Input: dimensioned drawing with shaded views. Units: mm. Origin: part minimum x, y, z. A direction names the side the tool comes from. Coordinates: 2 decimals unless noted, no trailing zeros. Order: outer loops, then holes, each group sorted by start corner. A loop starts at its lowest first (then second) coordinate and runs counter-clockwise, first axis right, second up. Notation, with made-up numbers: (-4, 36.5) - (19, 36.5) arc R20 ccw to (19, 74.5) - close; hole circle Ø4 at (6.5, 18). An arc over 180 degrees is marked (long way). Answer as CSV lines item,"result". Start each with the question number.
Item 1: Section C-C (x = 9). Output: boundary loops of the cut face in (y, z), and give its area (3 significant figures).
Item 2: Material intervals for line 1 along Z through (x, y) = (21, 7) (1 decimal); line 2 along Z through (x, y) = (38, 8) (1 decimal); line 3 along Y through (x, z) = (31.5, 28) (1 decimal), sorted ascending.
Item 3: Section A-A (x = 30). Output: boundary loops of the cut face in (y, z) (1 decimal), and give its area (3 significant figures).
Item 4: Section B-B (x = 4). Output: boundary loops of the cut face in (y, z) (1 decimal), and give its area (3 significant figures).
Item 5: First-contact query: pin 1 (6 mm diameter, centred on x = 35.5, y = 13, fed in from -Z); pin 2 (12 mm diameter, centred on x = 33, z = 17.5, fed in from -Y); pin 3 (3 mm diameter, centred on x = 23.5, z = 29, fed in from -Y) (1 decimal). Flat tips, straight axial feed; report the tip coordinate or a pass-through.
Item 6: Access query for the marked faces 1, 2, 3, 4 and 5. Directions: +Z, -Z, +X, -X, +Y, -Y. A direction counts if a zero-diameter tool reaches every point of the face in a straight line with its end or side. Return the directions, or none.
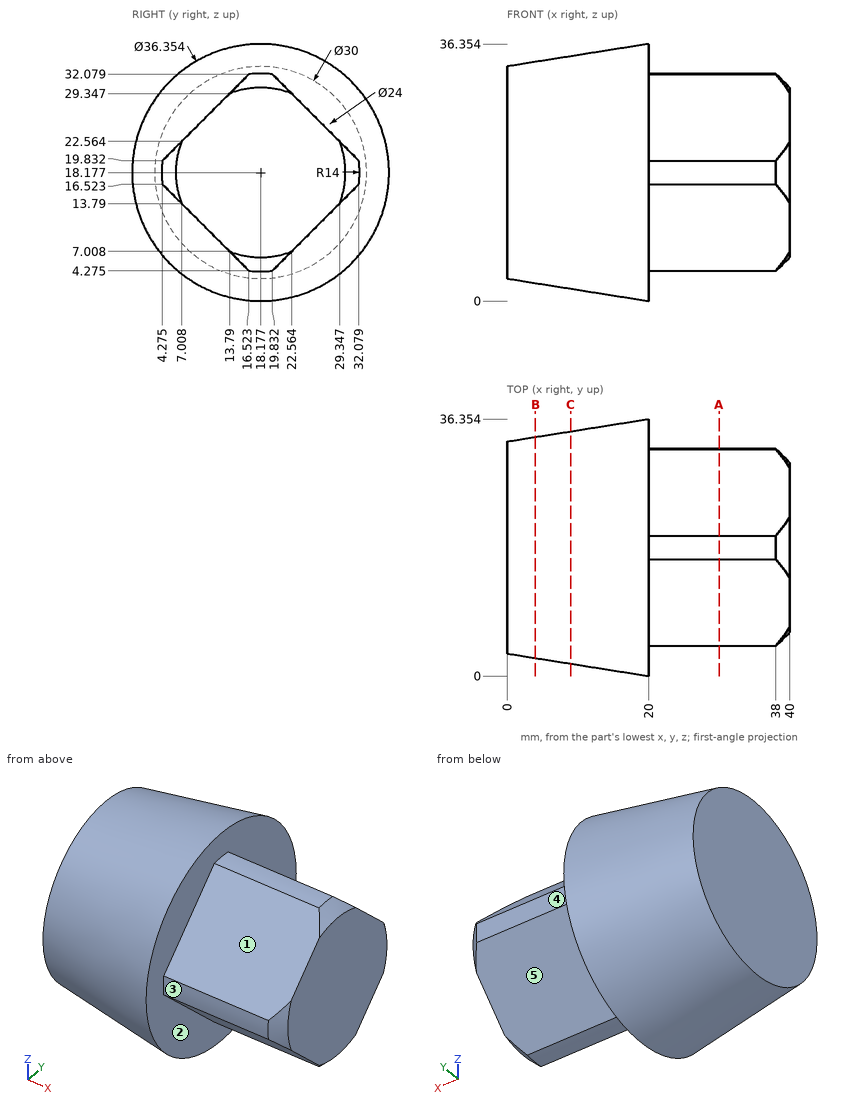
Determined:
1,outline,"circle Ø32.86 at (18.18, 18.18)"
1,area,"848 mm^2"
2,line 1,"z = 13.8 to 22.6"
2,line 2,"z = 12.8 to 23.6"
2,line 3,"y = 12.4 to 23.9"
3,outline,"(4.3, 16.5) - (16.5, 4.3) arc R14 ccw to (19.8, 4.3) - (32.1, 16.5) arc R14 ccw to (32.1, 19.8) - (19.8, 32.1) arc R14 ccw to (16.5, 32.1) - (4.3, 19.8) arc R14 ccw to start"
3,area,"474 mm^2"
4,outline,"circle Ø31.3 at (18.2, 18.2)"
4,area,"768 mm^2"
5,pin 1,"stops at z = 4.8"
5,pin 2,"stops at y = 4.18"
5,pin 3,"stops at y = 11.9"
6,face 1,"+Z, +X, -Y"
6,face 2,"+X"
6,face 3,"+X, -Y"
6,face 4,"+X, +Y"
6,face 5,"-Z, +X, +Y"
